Geometry check sheet. Reference: the model listing, model coordinates, mm. Face numbers are marked on the shaded views. Round coordinates to 2 decimals unless told otherwise and drop trailing zeros. Write each loop counter-clockwise with the first axis right and the second up, starting at its lowest first coordinate (ties: lowest second). Pieces come first, ordered by that corner, then holes.
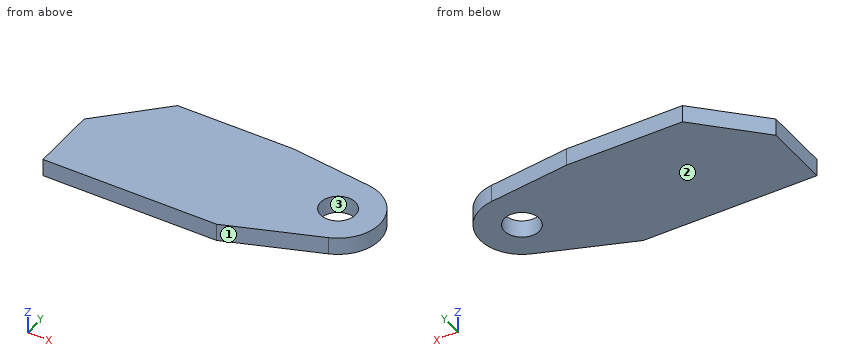
from build123d import *

# Parameters (mm, degrees)
SKETCH1_R           = 30
BOSS_EXTRUDE1_DEPTH = 30


with BuildPart() as part:
    # Sketch1 → Boss-Extrude1 (new body)
    with BuildSketch(Plane.XY):
        with BuildLine():
            Line((0, 0), (300, 0))
            Line((300, 0), (457.131807961, 58.528582136))
            ThreePointArc((457.131807961, 58.528582136), (503.513512073, 134.355692129), (440.900386954, 197.44776492))
            Line((440.900386954, 197.44776492), (300, 215))
            Line((300, 215), (100, 215))
            Line((100, 215), (0, 115))
            Line((0, 115), (0, 0))
        make_face()
        with Locations((432, 126)):
            Circle(SKETCH1_R, mode=Mode.SUBTRACT)
    extrude(amount=BOSS_EXTRUDE1_DEPTH)


solid = part.part
1. Scan lines: line 1 along X through (y, z) = (128, 28.75); line 2 along X through (y, z) = (146.5, 27); line 3 along Y through (x, z) = (437, 4.5). Record each from-to range of solid material in increasing order.
2. Section check C-C (x = 432). Record the cut outline in (y, z).
3. Depth check by flat-ended pin: pin 1 Ø5 at (x, z) = (385, 14.5) entering from -Y; pin 2 Ø4 at (y, z) = (114, 24) entering from +X. Enter the tip coordinate at first touch or a pass-through.
4. Section check A-A (y = 126). Record the cut outline in (x, z).
5. Release check for a two-part mould opening along Y. For the marked faces 1, 2 and 3 record: +Y half, -Y half, draft (parallel to the pull), parting line (faces both ways), or undercut.
6. Section check B-B (z = 24.75). Record the cut outline in (x, y).
7. Section check D-D (x = 325.5). Record the cut outline in (y, z), plus the area to 3 significant figures.
Results below:
1. line 1: x = 13 to 402.07, 461.93 to 503.97
1. line 2: x = 31.5 to 410.1, 453.9 to 501.02
1. line 3: y = 51.03 to 96.42, 155.58 to 197.93
2. outline: (49.17, 0) - (96, 0) - (96, 30) - (49.17, 30) - close; (156, 0) - (198.56, 0) - (198.56, 30) - (156, 30) - close
3. pin 1: stops at y = 30.73
3. pin 2: stops at x = 503.3
4. outline: (11, 0) - (402, 0) - (402, 30) - (11, 30) - close; (462, 0) - (504, 0) - (504, 30) - (462, 30) - close
5. face 1: -Y half
5. face 2: draft
5. face 3: undercut
6. outline: (0, 0) - (300, 0) - (457.13, 58.53) arc R72 ccw to (440.9, 197.45) - (300, 215) - (100, 215) - (0, 115) - close; hole circle Ø60 at (432, 126)
7. outline: (9.5, 0) - (211.82, 0) - (211.82, 30) - (9.5, 30) - close
7. area: 6,070 mm2
